For this review, use the dimensioned drawing (mm, ordinates from the lowest corner) and the shaded views. A direction names the side the tool comes from. Round coordinates to 2 decimals unless told otherwise and drop trailing zeros. Write each loop counter-clockwise with the first axis right and the second up, starting at its lowest first coordinate (ties: lowest second). Pieces come first, ordered by that corner, then holes. Notation, with made-up numbers: (48, -37.5) - (60, -37.5) arc R38 ccw to (60, 0.5) - close; hole circle Ø8 at (25, 79). An arc over 180 degrees is marked (long way). Return JSON: item names as keys, results as strings.
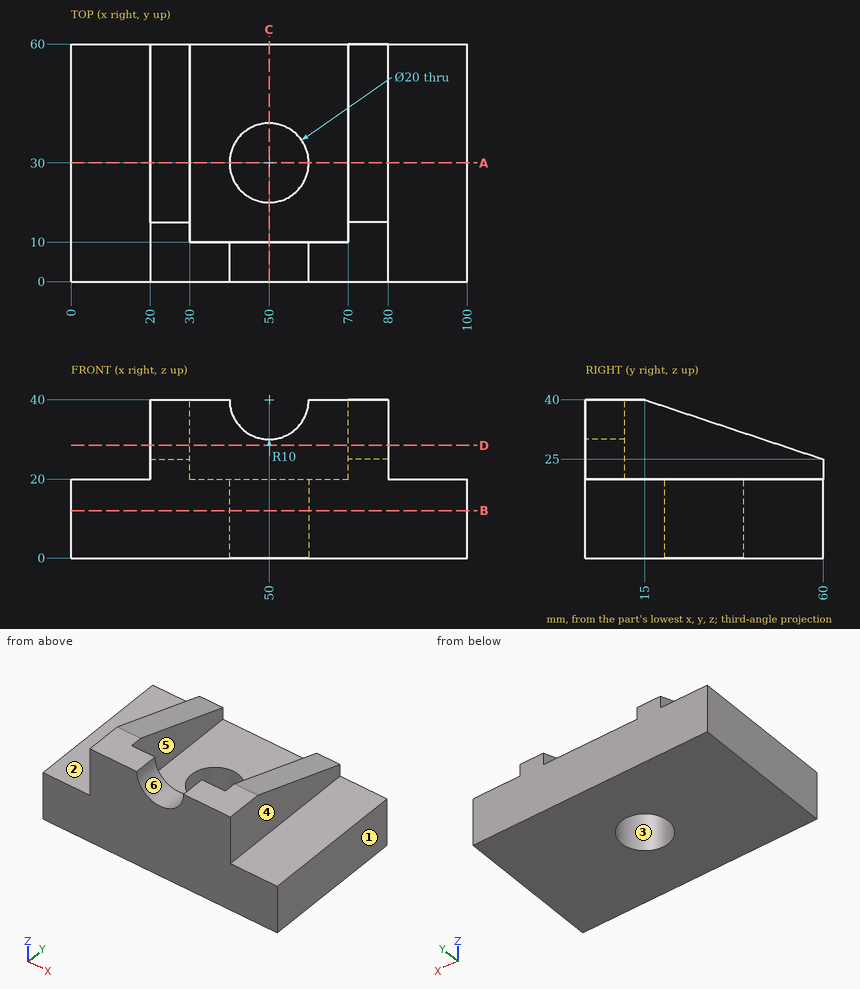
(1) For the marked faces 4, 5 and 6, list the 3-axis set-ups (+Z, -Z, +X, -X, +Y, -Y) from which the entire face can be reached by the end or side of a thin tool; tool diameter is ignored.
Filled in:
{"face 4": "+Z, +X, +Y, -Y", "face 5": "+Z, +Y", "face 6": "+Z, +Y, -Y"}
(2) Add section A-A (y = 30). Write out the cut boundary in (x, z), plus the area to 3 significant figures.
Filled in:
{"outline": "(0, 0) - (40, 0) - (40, 20) - (30, 20) - (30, 35) - (20, 35) - (20, 20) - (0, 20) - close; (60, 0) - (100, 0) - (100, 20) - (80, 20) - (80, 35) - (70, 35) - (70, 20) - (60, 20) - close", "area": "1,900 mm2"}
(3) Wall thickness on line 1 (Y direction, x = 50, z = 7); line 2 (X direction, y = 15.5, z = 26.5); line 3 (Z direction, x = 33, y = 19): over which ranges is each line inside the solid? List them lowest first.
Filled in:
{"line 1": "y = 0 to 20, 40 to 60", "line 2": "x = 20 to 30, 70 to 80", "line 3": "z = 0 to 20"}
(4) Add section D-D (z = 28.5). Write out the cut boundary in (x, y).
Filled in:
{"outline": "(20, 0) - (80, 0) - (80, 49.5) - (70, 49.5) - (70, 10) - (30, 10) - (30, 49.5) - (20, 49.5) - close"}
(5) Add section B-B (z = 12). Write out the cut boundary in (x, y).
Filled in:
{"outline": "(0, 0) - (100, 0) - (100, 60) - (0, 60) - close; hole circle Ø20 at (50, 30)"}
(6) Add section C-C (x = 50). Write out the cut boundary in (y, z), plus the area to 3 significant figures.
Filled in:
{"outline": "(0, 0) - (20, 0) - (20, 20) - (10, 20) - (10, 30) - (0, 30) - close; (40, 0) - (60, 0) - (60, 20) - (40, 20) - close", "area": "900 mm2"}
(7) Mouldability with a two-part tool opening along X and no side actions: class the marked faces 1, 2 and 3 as released by +X, released by -X, zero draft, split by the parting line, or undercut.
Filled in:
{"face 1": "released by +X", "face 2": "zero draft", "face 3": "undercut"}
(8) Clearance check with flat-ended pins moving along their axes: pin 1 Ø16 at (x, y) = (6, 40.5) entering from +Z; pin 2 Ø16 at (x, z) = (42.5, 31.5) entering from +Y; pin 3 Ø2 at (y, z) = (50, 21.5) entering from -X. State where each tip first meets the part, or that it passes through.
Filled in:
{"pin 1": "stops at z = 20", "pin 2": "stops at y = 10", "pin 3": "stops at x = 20"}
